```python
from build123d import *

# Parameters (mm, degrees)
EXTRUDE_1_DEPTH          = 20.5
EXTRUDE_START            = -3
EXTRUDE_2_DEPTH          = 3
EXTRUDE_START_2          = -2
EXTRUDE_3_DEPTH          = 2
CUT_EXTRUDE_1_DEPTH      = 35
CUT_EXTRUDE_1_DEPTH_BACK = 35
SKETCH_4_W               = 40
SKETCH_4_H               = 35
SKETCH_6_W               = 9.9
SKETCH_6_H               = 24
SKETCH_7_W               = 9.9
SKETCH_7_H               = 2
CUT_EXTRUDE_2_DEPTH      = 20
CUT_EXTRUDE_2_DEPTH_BACK = 20
SKETCH_8_W               = 3.6
SKETCH_8_H               = 1
SKETCH_10_W              = 1.5
SKETCH_10_H              = 5
EXTRUDE_4_DEPTH          = 11.5
EXTRUDE_4_DEPTH_BACK     = 11.5
SKETCH_12_W              = 23
SKETCH_12_H              = 9
CUT_EXTRUDE_3_DEPTH      = 0.3


with BuildPart() as part:
    # 草图1 → 凸台-拉伸1 (new body)
    with BuildSketch(Plane(origin=(0, -9, 0), x_dir=(-1, 0, 0), z_dir=(0, 1, 0))):
        with BuildLine():
            Line((16.5, -12.913670522), (16.5, 26.913670522))
            ThreePointArc((16.5, 26.913670522), (16.059625735, 28.165695908), (14.932432432, 28.866361535))
            ThreePointArc((14.932432432, 28.866361535), (0, 30.5), (-14.932432432, 28.866361535))
            ThreePointArc((-14.932432432, 28.866361535), (-16.059625735, 28.165695908), (-16.5, 26.913670522))
            Line((-16.5, 26.913670522), (-16.5, -12.913670522))
            ThreePointArc((-16.5, -12.913670522), (-16.059625735, -14.165695908), (-14.932432432, -14.866361535))
            ThreePointArc((-14.932432432, -14.866361535), (0, -16.5), (14.932432432, -14.866361535))
            ThreePointArc((14.932432432, -14.866361535), (16.059625735, -14.165695908), (16.5, -12.913670522))
        make_face()
    extrude(amount=EXTRUDE_1_DEPTH)

    # 草图2 → 凸台-拉伸2 (add)
    with BuildSketch(Plane(origin=(0, -9, 0), x_dir=(-1, 0, 0), z_dir=(0, 1, 0)).offset(EXTRUDE_START)):
        with BuildLine():
            Line((16.5, -12.913670522), (16.5, 26.913670522))
            ThreePointArc((16.5, 26.913670522), (16.059625735, 28.165695908), (14.932432432, 28.866361535))
            ThreePointArc((14.932432432, 28.866361535), (0, 30.5), (-14.932432432, 28.866361535))
            ThreePointArc((-14.932432432, 28.866361535), (-16.059625735, 28.165695908), (-16.5, 26.913670522))
            Line((-16.5, 26.913670522), (-16.5, -12.913670522))
            ThreePointArc((-16.5, -12.913670522), (-16.059625735, -14.165695908), (-14.932432432, -14.866361535))
            ThreePointArc((-14.932432432, -14.866361535), (0, -16.5), (14.932432432, -14.866361535))
            ThreePointArc((14.932432432, -14.866361535), (16.059625735, -14.165695908), (16.5, -12.913670522))
        make_face()
    extrude(amount=EXTRUDE_2_DEPTH)

    # 草图3 → 凸台-拉伸3 (add)
    with BuildSketch(Plane(origin=(0, -12, 0), x_dir=(-1, 0, 0), z_dir=(0, 1, 0)).offset(EXTRUDE_START_2)):
        with BuildLine():
            Line((16.5, -12.913670522), (16.5, 26.913670522))
            ThreePointArc((16.5, 26.913670522), (16.059625735, 28.165695908), (14.932432432, 28.866361535))
            ThreePointArc((14.932432432, 28.866361535), (0, 30.5), (-14.932432432, 28.866361535))
            ThreePointArc((-14.932432432, 28.866361535), (-16.059625735, 28.165695908), (-16.5, 26.913670522))
            Line((-16.5, 26.913670522), (-16.5, -12.913670522))
            ThreePointArc((-16.5, -12.913670522), (-16.059625735, -14.165695908), (-14.932432432, -14.866361535))
            ThreePointArc((-14.932432432, -14.866361535), (0, -16.5), (14.932432432, -14.866361535))
            ThreePointArc((14.932432432, -14.866361535), (16.059625735, -14.165695908), (16.5, -12.913670522))
        make_face()
    extrude(amount=EXTRUDE_3_DEPTH)

    # 草图4 → 切除-拉伸1 (cut, two sides: drawn at the far end of the back side and taken through both)
    with BuildSketch(Plane.XY.offset(-CUT_EXTRUDE_1_DEPTH_BACK)):
        with Locations((0, -2.5)):
            Rectangle(SKETCH_4_W, SKETCH_4_H)
        with BuildLine():
            Line((-16.5, 9.5), (-16.5, -12))
            ThreePointArc((-16.5, -12), (-15.914213562, -13.414213562), (-14.5, -14))
            Line((-14.5, -14), (14.5, -14))
            ThreePointArc((14.5, -14), (15.914213562, -13.414213562), (16.5, -12))
            Line((16.5, -12), (16.5, 9.5))
            ThreePointArc((16.5, 9.5), (15.914213562, 10.914213562), (14.5, 11.5))
            Line((14.5, 11.5), (-14.5, 11.5))
            ThreePointArc((-14.5, 11.5), (-15.914213562, 10.914213562), (-16.5, 9.5))
        make_face(mode=Mode.SUBTRACT)
    extrude(amount=CUT_EXTRUDE_1_DEPTH + CUT_EXTRUDE_1_DEPTH_BACK, mode=Mode.SUBTRACT)

    # 草图6 → 切除-旋转1 (revolve, cut)
    with BuildSketch(Plane(origin=(0, 0, 0), x_dir=(0, 0, -1), z_dir=(1, 0, 0))):
        with Locations((-4.95, 0)):
            Rectangle(SKETCH_6_W, SKETCH_6_H)
    revolve(axis=Axis((0, 12, 0), (0, -1, 0)), mode=Mode.SUBTRACT)

    # 草图7 → 切除-旋转2 (revolve, cut)
    with BuildSketch(Plane(origin=(0, 0, 0), x_dir=(0, 0, -1), z_dir=(1, 0, 0))):
        with Locations((-4.95, -13)):
            Rectangle(SKETCH_7_W, SKETCH_7_H)
    revolve(axis=Axis((0, -12, 0), (0, -1, 0)), mode=Mode.SUBTRACT)

    # 草图9 → 切除-拉伸2 (cut, two sides: drawn at the far end of the back side and taken through both)
    with BuildSketch(Plane(origin=(0, 0, 0), x_dir=(0, 0, -1), z_dir=(1, 0, 0)).offset(-CUT_EXTRUDE_2_DEPTH_BACK)):
        with BuildLine():
            Line((-35, -25), (-15, -25))
            Line((-15, -25), (-15, -14))
            Line((-15, -14), (-30.5, -14))
            Line((-30.5, -14), (-30.5, -3.888417686))
            Line((-30.5, -3.888417686), (-25.949027977, 10.118033989))
            ThreePointArc((-25.949027977, 10.118033989), (-25.222485449, 11.118033989), (-24.046914944, 11.5))
            Line((-24.046914944, 11.5), (-15, 11.5))
            Line((-15, 11.5), (-15, 25))
            Line((-15, 25), (-35, 25))
            Line((-35, 25), (-35, -25))
        make_face()
    extrude(amount=CUT_EXTRUDE_2_DEPTH + CUT_EXTRUDE_2_DEPTH_BACK, mode=Mode.SUBTRACT)

    # 草图8 → 旋转1 (revolve)
    with BuildSketch(Plane(origin=(0, 0, 0), x_dir=(0, 0, -1), z_dir=(1, 0, 0))):
        with Locations((-11.7, 11.5)):
            Rectangle(SKETCH_8_W, SKETCH_8_H)
    revolve(axis=Axis((0, 5, 0), (0, -1, 0)))

    # 草图5 → 旋转2 (revolve)
    with BuildSketch(Plane(origin=(0, 0, 0), x_dir=(0, 0, -1), z_dir=(1, 0, 0))):
        Polygon((-22, -17), (-24.7, -17), (-25, -16.7), (-25, -10), (-22, -10), align=None)
    revolve(axis=Axis((0, -10, 22), (0, -1, 0)))

    # 草图10 → 切除-旋转3 (revolve, cut)
    with BuildSketch(Plane(origin=(0, 0, 0), x_dir=(0, 0, -1), z_dir=(1, 0, 0)), mode=Mode.PRIVATE) as cut_revolve_3_sk:
        with Locations((-21.25, -14.5)):
            Rectangle(SKETCH_10_W, SKETCH_10_H)
    revolve(cut_revolve_3_sk.sketch.rotate(Axis((0, -17, 22), (0, 1, 0)), 180), axis=Axis((0, -17, 22), (0, 1, 0)), mode=Mode.SUBTRACT)

    # 草图11 → 凸台-拉伸4 (add, two sides: drawn at the far end of the back side and taken through both)
    with BuildSketch(Plane(origin=(0, 0, 0), x_dir=(0, 0, -1), z_dir=(1, 0, 0)).offset(-EXTRUDE_4_DEPTH_BACK)):
        with BuildLine():
            Line((-28.586737114, 2), (-26, 2))
            Line((-26, 2), (-26, 8))
            Line((-26, 8), (-26.637218937, 8))
            ThreePointArc((-26.637218937, 8), (-28.326233362, 5.232075627), (-28.586737114, 2))
        make_face()
    extrude(amount=EXTRUDE_4_DEPTH + EXTRUDE_4_DEPTH_BACK)

    # 草图12 → 切除-拉伸3 (cut)
    with BuildSketch(Plane(origin=(0, 11.5, 0), x_dir=(-1, 0, 0), z_dir=(0, 1, 0))):
        with Locations((0, 18)):
            Rectangle(SKETCH_12_W, SKETCH_12_H)
    extrude(amount=-CUT_EXTRUDE_3_DEPTH, mode=Mode.SUBTRACT)


solid = part.part
```
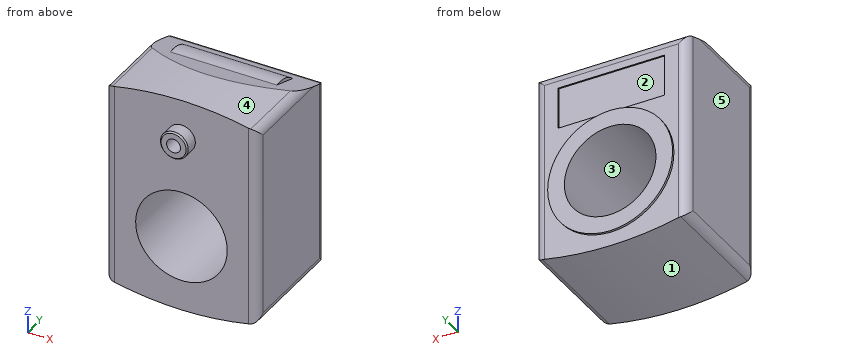
Source: CAD feature listing. Evaluate the final solid. Frame: model axes, mm. Face numbers are marked on the shaded views. A direction names the side the tool comes from. Give positions to 0.01 mm unless a question says otherwise; leave off trailing zeros. Loops run counter-clockwise (first coordinate to the right, second up) from the corner with the lowest first, then second, coordinate; pieces in that order, holes last. Notation, with made-up numbers: (29.25, -16) - (79.25, -16) arc R14 ccw to (79.25, 0) - close; hole circle Ø1 at (-5, 40). An arc over 180 degrees is marked (long way). Use CSV: the item, a comma, the result in double quotes.
1) Pin query (flat end, axial travel): P1, Ø10, axis at x = -2, z = 19, coming from the +Y side; P2, Ø5, axis at x = -8.5, y = -8.5, coming from the +Z side; P3, Ø8, axis at x = -1.5, y = -3, coming from the +Z side; P4, Ø2.5, axis at x = 0, z = 22, coming from the -Y side. Return the tip coordinate at first contact, or that it passes through.
Worked out:
P1,"stops at y = 11.5"
P2,"stops at z = 30.24"
P3,"stops at z = 30.5"
P4,"stops at y = -12"
2) Cut plane B-B (y = -10.5). Output: boundary loops of the cut face in (x, z) (1 decimal).
Worked out:
outline,"(-16.5, -12.9) arc R2 ccw to (-14.9, -14.9) arc R69.1 ccw to (14.9, -14.9) arc R2 ccw to (16.5, -12.9) - (16.5, 26.9) arc R2 ccw to (14.9, 28.9) arc R69.1 ccw to (-14.9, 28.9) arc R2 ccw to (-16.5, 26.9) - close; hole circle Ø19.8 at (0, 0)"
3) Line query: line 1 (X direction, y = -15.65, z = 22); line 2 (X direction, y = 0.5, z = 0); line 3 (Y direction, x = -14, z = -14). Output: solid intervals per line, ascending.
Worked out:
line 1,"x = -3 to -1.5, 1.5 to 3"
line 2,"x = -16.5 to -9.9, 9.9 to 16.5"
line 3,"y = -14 to 11.5"
4) Set-up query: the marked faces 1 and 2. Return all of +Z, -Z, +X, -X, +Y, -Y with unobstructed straight access to the full face (end or side cutting, diameter ignored); none if empty.
Worked out:
face 1,"-Z, +Y, -Y"
face 2,"+Y"
5) Cut plane D-D (z = -11.5). Output: boundary loops of the cut face in (x, y), and give its area (3 significant figures).
Worked out:
outline,"(-16.5, -12) arc R2 ccw to (-14.5, -14) - (14.5, -14) arc R2 ccw to (16.5, -12) - (16.5, 9.5) arc R2 ccw to (14.5, 11.5) - (7.07, 11.5) - (7.07, 12) - (-7.07, 12) - (-7.07, 11.5) - (-14.5, 11.5) arc R2 ccw to (-16.5, 9.5) - close"
area,"845 mm^2"
6) Mould query, pull axis Z, two halves, no side actions, for the marked faces 3, 4 and 5. Classes: +Z half, -Z half, draft (parallel to the pull), parting line (faces both ways), or undercut.
Worked out:
face 3,"undercut"
face 4,"+Z half"
face 5,"draft"
7) Cut plane C-C (x = 5). Output: boundary loops of the cut face in (y, z).
Worked out:
outline,"(-14, -16.32) - (11.5, -16.32) - (11.5, -12.54) - (12, -12.54) - (12, -8.54) - (-14, -8.54) - close; (-14, 8.54) - (12, 8.54) - (12, 12.54) - (11.5, 12.54) - (11.5, 13.5) - (11.2, 13.5) - (11.2, 22.5) - (11.5, 22.5) - (11.5, 24.05) arc R2 ccw to (10.12, 25.95) - (8, 26.64) arc R7 ccw to (2, 28.59) - (-3.33, 30.32) - (-14, 30.32) - close"
8) Cut plane A-A (z = 0). Output: boundary loops of the cut face in (x, y).
Worked out:
outline,"(-16.5, -12) arc R2 ccw to (-14.5, -14) - (-9.9, -14) - (-9.9, 12) - (-13.5, 12) - (-13.5, 11.5) - (-14.5, 11.5) arc R2 ccw to (-16.5, 9.5) - close; (9.9, -14) - (14.5, -14) arc R2 ccw to (16.5, -12) - (16.5, 9.5) arc R2 ccw to (14.5, 11.5) - (13.5, 11.5) - (13.5, 12) - (9.9, 12) - close"
